Build history of the part. All positions in model axes, mm. A direction names the side the tool comes from. Round coordinates to 2 decimals unless told otherwise and drop trailing zeros. Write each loop counter-clockwise with the first axis right and the second up, starting at its lowest first coordinate (ties: lowest second). Pieces come first, ordered by that corner, then holes. Notation, with made-up numbers: M 61,-31 L 72,-31 A20 cw 72,-24 Z; hole C 50,38 d1. An arc over 180 degrees is marked long. Write item = value, one per line. Start each with the question number.
Q1. Band-saw the part on D-D on y = 65. Write the cut outline in (x, z).
Q2. Band-saw the part on C-C on z = 33.5. Write the cut outline in (x, y).
Q3. Drop flat-ended pins along their axis: P1, Ø6, axis at y = 55, z = 28, coming from the -X side; P2, Ø7, axis at y = 63, z = 23, coming from the +X side; P3, Ø14.5, axis at y = 30, z = 9.5, coming from the -X side. Give the stop position or say it passes through.
Q4. Tool access for faces 4 (the flat face through (-28.708, 32, 0)), 5 (the cylindrical face through (13.843, -26.615, 0.56)), 6 (the flat face through (-28, 51, -30)), 7 (the flat face through (8.5, 46.1, 0.1)), 8 (the flat face through (-28, 51, 30)): list every direction of +Z, -Z, +X, -X, +Y, -Y with a clear straight run to the whole face (end or side of a thin tool).
Q5. Band-saw the part on B-B on x = 0. Write the cut outline in (y, z).
Q6. Band-saw the part on A-A on y = 0. Write the cut outline in (x, z).
Q7. Pull direction Y, two halves, no side cores. Call faces 1 (the flat face through (-63.4, 116.708, -9.2)), 2 (the cylindrical face through (-14.985, 0.66, -0.56)), 3 (the cylindrical face through (-67.946, 87.128, -3.83)): released by +Y, released by -Y, zero draft, split by the parting line, or undercut.
Q8. Probe L1, parallel to Y at x = 0, z = 24.5; L2, parallel to Y at x = -8.5, z = 18; L3, parallel to X at y = 92, z = -2. List the from-to ranges inside material, lowest first.
```python
from build123d import *

# Parameters (mm, degrees)
BASE_BLOCK_SKETCH_R            = 30
BASE_BLOCK_SKETCH_R_2          = 15
BASE_BLOCK_DEPTH               = 40
ARM_DEPTH                      = 30
SUPPORT_RIB_DEPTH              = 6
PROFILE_CUT_DEPTH              = 145.415437787
DRAFTED_BOSS_SKETCH_R          = 30
DRAFTED_CYLINDRICAL_BOSS_DEPTH = 40
DRAFTED_CYLINDRICAL_BOSS_TAPER = 14
BOSS_BORE_SKETCH_R             = 10
BOSS_BORE_20_DEPTH             = 177.046816624


with BuildPart() as part:
    # Base Block Sketch → Base Block (new, symmetric)
    with BuildSketch(Plane.XY):
        Circle(BASE_BLOCK_SKETCH_R)
        Circle(BASE_BLOCK_SKETCH_R_2, mode=Mode.SUBTRACT)
    extrude(amount=BASE_BLOCK_DEPTH, both=True)

    # Arm Profile Sketch → Arm (add, symmetric)
    with BuildSketch(Plane.XY):
        with BuildLine():
            Line((-28.708286934, 8.708286934), (-28.708286934, 56.708286934))
            Line((-28.708286934, 56.708286934), (-88.708286934, 56.708286934))
            Line((-88.708286934, 56.708286934), (-88.708286934, 76.708286934))
            Line((-88.708286934, 76.708286934), (-8.708286934, 76.708286934))
            Line((-8.708286934, 76.708286934), (-8.708286934, 28.708286934))
            ThreePointArc((-8.708286934, 28.708286934), (-21.213203436, 21.213203436), (-28.708286934, 8.708286934))
        make_face()
    extrude(amount=ARM_DEPTH, both=True)

    # Support Rib Sketch → Support Rib (add, symmetric)
    with BuildSketch(Plane.XY):
        with BuildLine():
            Line((-8.708286934, 76.708286934), (26.150815657, 14.701525107))
            ThreePointArc((26.150815657, 14.701525107), (11.185159645, 27.836885668), (-8.708286934, 28.708286934))
            Line((-8.708286934, 28.708286934), (-8.708286934, 76.708286934))
        make_face()
    extrude(amount=SUPPORT_RIB_DEPTH, both=True)

    # Profile Cut Sketch → Profile Cut (cut, through all)
    with BuildSketch(Plane(origin=(0, 76.708286934, 0), x_dir=(1, 0, 0), z_dir=(0, 1, 0))):
        with BuildLine():
            Line((-88.708286934, -30), (-58.708286934, -30))
            ThreePointArc((-58.708286934, -30), (-79.921490369, -21.213203436), (-88.708286934, 0))
            Line((-88.708286934, 0), (-88.708286934, -30))
        make_face()
        with BuildLine():
            ThreePointArc((-88.708286934, 0), (-79.921490369, 21.213203436), (-58.708286934, 30))
            Line((-58.708286934, 30), (-88.708286934, 30))
            Line((-88.708286934, 30), (-88.708286934, 0))
        make_face()
    extrude(amount=-PROFILE_CUT_DEPTH, mode=Mode.SUBTRACT)

    # Drafted Boss Sketch → Drafted Cylindrical Boss (add)
    with BuildSketch(Plane(origin=(0, 76.708286934, 0), x_dir=(1, 0, 0), z_dir=(0, 1, 0))):
        with Locations((-58.708286934, 0)):
            Circle(DRAFTED_BOSS_SKETCH_R)
    extrude(amount=DRAFTED_CYLINDRICAL_BOSS_DEPTH, taper=DRAFTED_CYLINDRICAL_BOSS_TAPER)

    # Boss Bore Sketch → Boss Bore Ø20 (cut, through all)
    with BuildSketch(Plane(origin=(0, 116.708286934, 0), x_dir=(1, 0, 0), z_dir=(0, 1, 0))):
        with Locations(Location((-58.708286934, 0, 0), (0, 0, 180))):
            Circle(BOSS_BORE_SKETCH_R)
    extrude(amount=-BOSS_BORE_20_DEPTH, mode=Mode.SUBTRACT)


solid = part.part
```
Conclusion:
q1.outline = M -58.71,-30 L -8.71,-30 L -8.71,-6 L -2.13,-6 L -2.13,6 L -8.71,6 L -8.71,30 L -58.71,30 A30 ccw Z; hole C -58.71,0 d20
q2.outline = C 0,0 d60; hole C 0,0 d30
q3.P1 = -74.46
q3.P2 = -8.71
q3.P3 = -28.71
q4.face_4 = +Z, -Z, -X
q4.face_5 = none
q4.face_6 = -Z, -X, +Y
q4.face_7 = +Z, -Z, +X, +Y
q4.face_8 = +Z, -X, +Y
q5.outline = M -30,-40 L -15,-40 L -15,40 L -30,40 Z; M 15,-40 L 30,-40 L 30,-6 L 61.22,-6 L 61.22,6 L 30,6 L 30,40 L 15,40 Z
q6.outline = M -30,-40 L -15,-40 L -15,40 L -30,40 Z; M 15,-40 L 30,-40 L 30,40 L 15,40 Z
q7.face_1 = released by +Y
q7.face_2 = undercut
q7.face_3 = zero draft
q8.L1 = -30 to -15, 15 to 30
q8.L2 = -28.77 to -12.36, 12.36 to 28.77
q8.L3 = -84.82 to -68.51, -48.91 to -32.6
